The listing builds one solid part. Answer for the finished solid, in the listing's coordinates (mm). A direction names the side the tool comes from. Give positions to 0.01 mm unless a question says otherwise; leave off trailing zeros. Write each loop counter-clockwise with the first axis right and the second up, starting at its lowest first coordinate (ties: lowest second). Pieces come first, ordered by that corner, then holes. Notation, with made-up numbers: (-0.5, -12) - (10.5, -12) arc R23 cw to (10.5, 10) - close; hole circle Ø6 at (46.25, 0.5). An arc over 180 degrees is marked (long way). Use a Markdown table: item, result. Add a question column.
from build123d import *

# Parameters (mm, degrees)
SKETCH_1_R          = 12.5
EXTRUDE_1_DEPTH     = 35
SKETCH_3_R          = 10
EXTRUDE_3_DEPTH     = 55
SKETCH_4_W          = 1.3
SKETCH_4_H          = 0.55
CUT_EXTRUDE_1_DEPTH = 94.259047818
EXTRUDE_START       = 15
SKETCH_6_R          = 10
EXTRUDE_4_DEPTH     = 15


with BuildPart() as part:
    # 草图1 → 凸台-拉伸1 (new, symmetric)
    with BuildSketch(Plane(origin=(0, 0, 0), x_dir=(0, 0, -1), z_dir=(1, 0, 0))):
        Circle(SKETCH_1_R)
    extrude(amount=EXTRUDE_1_DEPTH, both=True)

    # 草图3 → 凸台-拉伸3 (add)
    with BuildSketch(Plane(origin=(35, 0, 0), x_dir=(0, 0, -1), z_dir=(1, 0, 0))):
        Circle(SKETCH_3_R)
    extrude(amount=EXTRUDE_3_DEPTH)

    # 草图4 → 切除-旋转1 (revolve, cut)
    with BuildSketch(Plane(origin=(0, 0, 0), x_dir=(1, 0, 0), z_dir=(0, 1, 0)), mode=Mode.PRIVATE) as cut_revolve_1_sk:
        with Locations((-16.15, 12.225)):
            Rectangle(SKETCH_4_W, SKETCH_4_H)
        with Locations((16.15, 12.225)):
            Rectangle(SKETCH_4_W, SKETCH_4_H)
    revolve(cut_revolve_1_sk.sketch.rotate(Axis((0, 0, 0), (1, 0, 0)), 180), axis=Axis((0, 0, 0), (1, 0, 0)), mode=Mode.SUBTRACT)

    # 草图5 → 切除-拉伸1 (cut, through all)
    with BuildSketch(Plane(origin=(0, 8.5, 0), x_dir=(1, 0, 0), z_dir=(0, 1, 0))):
        with BuildLine():
            Line((-5, 4), (15, 4))
            ThreePointArc((15, 4), (19, 0), (15, -4))
            Line((15, -4), (-5, -4))
            ThreePointArc((-5, -4), (-9, 0), (-5, 4))
        make_face()
    extrude(amount=CUT_EXTRUDE_1_DEPTH, mode=Mode.SUBTRACT)

    # 草图6 → 凸台-拉伸4 (add)
    with BuildSketch(Plane.ZY.offset(35).offset(EXTRUDE_START)):
        with Locations(Location((0, 0, 0), (0, 0, 180))):
            Circle(SKETCH_6_R)
    extrude(amount=-EXTRUDE_4_DEPTH)


solid = part.part
1. Consider L1, parallel to X at y = 8.75, z = 2.75; L2, parallel to Z at x = 20.5, y = -3.75; L3, parallel to X at y = -10, z = 3.75. Determine where each line is inside the solid, lowest interval first. Write a range as [from, to].
2. For a pull along Z with two mould halves and no side action, classify faces 6 (the flat face through (5, 10, 4)), 7 (the flat face through (5, 10, -4)), 8 (the flat face through (35, 10.2, 0.1)), 9 (the cylindrical face through (-16.14, -10.08, 6.42)) as released by +Z, released by -Z, zero draft, split by the parting line, or undercut.
3. Given P1, Ø1, axis at x = 1, y = 11, coming from the -Z side; P2, Ø1.5, axis at x = 55.5, y = -0.5, coming from the -Z side; P3, Ø2, axis at x = -25.5, y = -2.5, coming from the -Z side, each flat-ended and moving along its own axis, determine where each tip first touches the part or whether it passes through.
4. The part is cut by section B-B (z = -2.25). Give the vertices of the cut face in (x, y), and give its area (3 significant figures).
5. Which of the six approach directions +Z, -Z, +X, -X, +Y, -Y give full straight-line access (tool end or side, diameter ignored) to faces 1 (the cylindrical face through (16.16, -11.94, 0.47)), 2 (the cylindrical face through (19, 10, 0)), 3 (the flat face through (90, 0, 0)), 4 (the cylindrical face through (62.11, -9.76, 2.17)), 5 (the cylindrical face through (-43, 0, 10))?
6. The part is cut by section D-D (x = 50.5). Give the vertices of the cut face in (y, z), and give its area (3 significant figures).
7. The part is cut by section A-A (y = 0). Give the vertices of the cut face in (x, z), and give its area (3 significant figures).
8. The part is cut by section C-C (x = -10.5). Give the vertices of the cut face in (y, z), and give its area (3 significant figures).
Check values:
| question | item | result |
|---|---|---|
| 1 | L1 | x = [-50, -7.9], [17.9, 90] |
| 1 | L2 | z = [-11.92, 11.92] |
| 1 | L3 | x = [-35, 35] |
| 2 | face 6 | undercut |
| 2 | face 7 | undercut |
| 2 | face 8 | zero draft |
| 2 | face 9 | split by the parting line |
| 3 | P1 | stops at z = -6.78 |
| 3 | P2 | stops at z = -10 |
| 3 | P3 | stops at z = -12.41 |
| 4 | outline | (-50, -9.74) - (-35, -9.74) - (-35, -12.3) - (-16.8, -12.3) - (-16.8, -11.74) - (-15.5, -11.74) - (-15.5, -12.3) - (15.5, -12.3) - (15.5, -11.74) - (16.8, -11.74) - (16.8, -12.3) - (35, -12.3) - (35, -9.74) - (90, -9.74) - (90, 9.74) - (35, 9.74) - (35, 12.3) - (18.31, 12.3) - (18.31, 8.5) - (-8.31, 8.5) - (-8.31, 12.3) - (-15.5, 12.3) - (-15.5, 11.74) - (-16.8, 11.74) - (-16.8, 12.3) - (-35, 12.3) - (-35, 9.74) - (-50, 9.74) - close |
| 4 | area | 2,980 mm2 |
| 5 | face 1 | none |
| 5 | face 2 | +Y |
| 5 | face 3 | +Z, -Z, +X, +Y, -Y |
| 5 | face 4 | +X |
| 5 | face 5 | -X |
| 6 | outline | circle Ø20 at (0, 0) |
| 6 | area | 314 mm2 |
| 7 | outline | (-50, -10) - (-35, -10) - (-35, -12.5) - (-16.8, -12.5) - (-16.8, -11.95) - (-15.5, -11.95) - (-15.5, -12.5) - (15.5, -12.5) - (15.5, -11.95) - (16.8, -11.95) - (16.8, -12.5) - (35, -12.5) - (35, -10) - (90, -10) - (90, 10) - (35, 10) - (35, 12.5) - (16.8, 12.5) - (16.8, 11.95) - (15.5, 11.95) - (15.5, 12.5) - (-15.5, 12.5) - (-15.5, 11.95) - (-16.8, 11.95) - (-16.8, 12.5) - (-35, 12.5) - (-35, 10) - (-50, 10) - close |
| 7 | area | 3,150 mm2 |
| 8 | outline | circle Ø25 at (0, 0) |
| 8 | area | 491 mm2 |
